```python
from build123d import *

# Parameters (mm, degrees)
BASE_PLATE_SKETCH_W          = 65
BASE_PLATE_SKETCH_H          = 48
BASE_PLATE_DEPTH             = 12
UPPER_BLOCK_DEPTH            = 12
SUPPORT_WEB_SKETCH_R         = 10
SUPPORT_WEB_DEPTH            = 48
TOP_SLOT_SKETCH_W            = 16
TOP_SLOT_SKETCH_H            = 60
TOP_SLOT_DEPTH               = 3
HUB_BOSS_SKETCH_W            = 52
HUB_BOSS_SKETCH_H            = 60
HUB_BOSS_SKETCH_R            = 6
HUB_BOSS_DEPTH               = 12
HUB_ROUND_R30_R              = 30
UPPER_MOUNTING_HOLE_SKETCH_R = 5
UPPER_MOUNTING_HOLE_DEPTH    = 12
BASE_MOUNTING_HOLE_SKETCH_R  = 5
BASE_MOUNTING_HOLE_DEPTH     = 12
UPPER_BLOCK_FILLET_R10_R     = 10
SIDE_SUPPORT_DEPTH           = 48
SIDE_RELIEF_CUT_DEPTH        = 48


with BuildPart() as part:
    # Base Plate Sketch → Base Plate (new body)
    with BuildSketch(Plane(origin=(0, 0, 0), x_dir=(1, 0, 0), z_dir=(0, 1, 0))):
        Rectangle(BASE_PLATE_SKETCH_W, BASE_PLATE_SKETCH_H)
    extrude(amount=BASE_PLATE_DEPTH)

    # Upper Block Sketch → Upper Block (add)
    with BuildSketch(Plane(origin=(0, 0, -24), x_dir=(-1, 0, 0), z_dir=(0, 0, -1))):
        with BuildLine():
            Line((32.5, 12), (32.5, 82))
            Line((32.5, 82), (-77.5, 82))
            Line((-77.5, 82), (-77.5, 55))
            Line((-77.5, 55), (-65.5, 55))
            Line((-65.5, 55), (-65.5, 50))
            ThreePointArc((-65.5, 50), (-45.466720109, 34.068374642), (-32.5, 12))
            Line((-32.5, 12), (32.5, 12))
        make_face()
    extrude(amount=-UPPER_BLOCK_DEPTH)

    # Support Web Sketch → Support Web (add)
    with BuildSketch(Plane.XY.offset(-12)):
        with BuildLine():
            Line((0.150648427, 82), (34.849351573, 82))
            ThreePointArc((34.849351573, 82), (17.5, 39), (0.150648427, 82))
        make_face()
        with Locations((17.5, 64)):
            Circle(SUPPORT_WEB_SKETCH_R, mode=Mode.SUBTRACT)
    extrude(amount=SUPPORT_WEB_DEPTH)

    # Top Slot Sketch → Top Slot (cut)
    with BuildSketch(Plane(origin=(0, 82, 0), x_dir=(1, 0, 0), z_dir=(0, 1, 0))):
        with Locations((17.5, -6)):
            Rectangle(TOP_SLOT_SKETCH_W, TOP_SLOT_SKETCH_H)
    extrude(amount=-TOP_SLOT_DEPTH, mode=Mode.SUBTRACT)

    # Hub Boss Sketch → Hub Boss (add)
    with BuildSketch(Plane(origin=(0, 82, 0), x_dir=(1, 0, 0), z_dir=(0, 1, 0))):
        with Locations((51.5, -6)):
            Rectangle(HUB_BOSS_SKETCH_W, HUB_BOSS_SKETCH_H)
        with Locations(Location((57.5, -12, 0), (0, 0, 270))):
            Circle(HUB_BOSS_SKETCH_R, mode=Mode.SUBTRACT)
    extrude(amount=-HUB_BOSS_DEPTH)

    # Hub Round R30
    hub_round_r30_edges = [part.edges().sort_by_distance(p)[0] for p in [
        (77.5, 76, 36),
    ]]
    fillet(hub_round_r30_edges, radius=HUB_ROUND_R30_R)

    # Upper Mounting Hole Sketch → Upper Mounting Hole (cut)
    with BuildSketch(Plane.XY.offset(-12)):
        with Locations((-22.5, 72)):
            Circle(UPPER_MOUNTING_HOLE_SKETCH_R)
    extrude(amount=-UPPER_MOUNTING_HOLE_DEPTH, mode=Mode.SUBTRACT)

    # Base Mounting Hole Sketch → Base Mounting Hole (cut)
    with BuildSketch(Plane(origin=(0, 12, 0), x_dir=(1, 0, 0), z_dir=(0, 1, 0))):
        with Locations(Location((-22.5, -14, 0), (0, 0, 270))):
            Circle(BASE_MOUNTING_HOLE_SKETCH_R)
    extrude(amount=-BASE_MOUNTING_HOLE_DEPTH, mode=Mode.SUBTRACT)

    # Upper Block Fillet R10
    upper_block_fillet_r10_edges = [part.edges().sort_by_distance(p)[0] for p in [
        (-32.5, 82, -18),
        (-32.5, 6, 24),
    ]]
    fillet(upper_block_fillet_r10_edges, radius=UPPER_BLOCK_FILLET_R10_R)

    # Side Support Sketch → Side Support (add)
    with BuildSketch(Plane.XY.offset(-12)):
        with BuildLine():
            Line((17.5, 12), (12.5, 12))
            Line((12.5, 12), (12.5, 39.505102572))
            ThreePointArc((12.5, 39.505102572), (17.5, 39), (22.5, 39.505102572))
            Line((22.5, 39.505102572), (22.5, 12))
            Line((22.5, 12), (17.5, 12))
        make_face()
    extrude(amount=SIDE_SUPPORT_DEPTH)

    # Side Relief Sketch → Side Relief Cut (cut)
    with BuildSketch(Plane(origin=(22.5, 0, 0), x_dir=(0, 0, -1), z_dir=(1, 0, 0))):
        Polygon((-36, 39.505102572), (-24, 12), (-36, 12), align=None)
    extrude(amount=-SIDE_RELIEF_CUT_DEPTH, mode=Mode.SUBTRACT)


solid = part.part
```
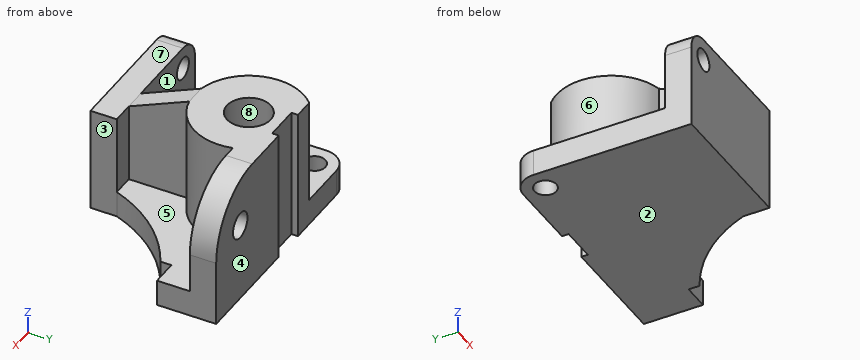
Build history of the part. All positions in model axes, mm. Face numbers are marked on the shaded views. A direction names the side the tool comes from. Give positions to 0.01 mm unless a question says otherwise; leave off trailing zeros. Loops run counter-clockwise (first coordinate to the right, second up) from the corner with the lowest first, then second, coordinate; pieces in that order, holes last.
Item 1: Pull direction X, two halves, no side cores. Call the marked faces 6, 7 and 8: released by +X, released by -X, zero draft, split by the parting line, or undercut.
Answers follow:
face 6: released by -X
face 7: zero draft
face 8: undercut
Item 2: Drill centre lines: line 1 (Y direction, x = -22.5, z = -17); line 2 (X direction, y = 64, z = 16); line 3 (Y direction, x = 32, z = 4.5). Where is each one in solid material? Low to high.
Answers follow:
line 1: y = 0 to 67, 77 to 82
line 2: x = -7.5 to 7.5, 27.5 to 42.5
line 3: y = 0 to 12, 43.63 to 82
Item 3: Slice it at C-C, the plane y = 7. List the corners of the cut face in (x, z).
Answers follow:
outline: (-32.5, -24) - (32.5, -24) - (32.5, 24) - (-22.5, 24) arc R10 ccw to (-32.5, 14) - close; hole circle Ø10 at (-22.5, 14)
Item 4: Slice it at B-B, the plane x = 57.5. List the corners of the cut face in (y, z).
Answers follow:
outline: (45.04, -24) - (82, -24) - (82, 6) - (70, 6) - (70, -12) - (45.04, -12) - close; (70, 18) - (82, 18) - (82, 34.28) - (70, 34.28) - close
Item 5: Slice it at D-D, the plane x = -12. List the corners of the cut face in (y, z).
Answers follow:
outline: (0, -24) - (82, -24) - (82, -12) - (12, -12) - (12, 24) - (0, 24) - close
Item 6: Flat gauge pins, fed straight in: pin 1 (10 mm diameter, centred on y = 56.5, z = 7, fed in from -X); pin 2 (1.5 mm diameter, centred on y = 81, z = -5, fed in from -X); pin 3 (3.5 mm diameter, centred on y = 6, z = -8.5, fed in from +X). Where does each tip first touch, or does it go through?
Answers follow:
pin 1: stops at x = -7.37
pin 2: stops at x = -1.5
pin 3: stops at x = 32.5
Item 7: Which spindle directions (+Z, -Z, +X, -X, +Y, -Y) get a long thin tool onto all of the face, cutting with end or side? Do the marked faces 1, 2, 3, 4 and 5. Say none if no direction does.
Answers follow:
face 1: +Z, -X
face 2: -Z, +X, -X, +Y, -Y
face 3: +Z, -Z, +X, -Y
face 4: +Z, -Z, +X, -X, +Y
face 5: +Z, +X
Item 8: Slice it at A-A, the plane z = -20. List the corners of the cut face in (x, y).
Answers follow:
outline: (-32.5, 0) - (32.5, 0) - (32.5, 12) arc R70 cw to (65.5, 50) - (65.5, 55) - (77.5, 55) - (77.5, 82) - (25.5, 82) - (25.5, 79) - (9.5, 79) - (9.5, 82) - (-22.5, 82) arc R10 ccw to (-32.5, 72) - close; hole circle Ø10 at (-22.5, 72)
